Verification items for the finished model (mm, model axes). A direction names the side the tool comes from. Round coordinates to 2 decimals unless told otherwise and drop trailing zeros. Order: outer loops, then holes, each group sorted by start corner. A loop starts at its lowest first (then second) coordinate and runs counter-clockwise, first axis right, second up. Notation, with made-up numbers: (74, 39) -> (114, 39) arc R21 cw to (114, 59) -> close; hole circle Ø4 at (15, 56.5). An arc over 180 degrees is marked (long way). Return JSON: item names as keys, results as strings. Group by question number.
Item 1: Access from +Z, -Z, +X, -X, +Y, -Y to the whole of each face (thin tool, end or side, straight path). Record for faces 1 (the flat face through (28, 122, 0)), 2 (the flat face through (29, 50, -6.5)), 3 (the flat face through (70, 0, -1)).
Item 2: Sectioned sample at A-A on y = 129. Record the cut outline in (x, z), plus the area to 4 significant figures.
Item 3: Sectioned sample at B-B on x = 15. Record the cut outline in (y, z).
Item 4: Sectioned sample at C-C on x = 132. Record the cut outline in (y, z).
Item 5: Depth check by flat-ended pin: pin 1 Ø2 at (y, z) = (38, 0.5) entering from +X; pin 2 Ø3 at (x, z) = (27.5, -1) entering from -Y; pin 3 Ø13.5 at (x, y) = (15, 129) entering from -Z; pin 4 Ø6 at (y, z) = (86.5, 4) entering from +X. Enter the tip coordinate at first touch or a pass-through.
Item 6: Sectioned sample at D-D on z = 1. Record the cut outline in (x, y), plus the area to 3 significant figures.
Item 7: Draft check along X on faces 4 (the cylindrical face through (137.495, 23.758, -0.091)), 5 (the cylindrical face through (2.281, 141.594, 0.091)), 6 (the flat face through (142, 12, 0)). Enter one of: pulls with the +X half, pulls with the -X half, needs draft (parallel to the pull), parting line crosses it, or undercut.
Item 8: Scan lines: probe 1 along Y at (x, z) = (15, -0.75); probe 2 along X at (y, z) = (24, 0.75); probe 3 along Y at (x, z) = (132, 1.75). Record each from-to range of solid material in increasing order. Write a range as from..to.
```python
from build123d import *

# Parameters (mm, degrees)
SKETCH1_R           = 5.5
BOSS_EXTRUDE1_DEPTH = 6.5
SKETCH2_W           = 142
SKETCH2_H           = 7
BOSS_EXTRUDE2_DEPTH = 3
M10_TAPPED_HOLE1_D  = 8.5
FILLET1_R           = 8


with BuildPart() as part:
    # Sketch1 → Boss-Extrude1 (new, symmetric)
    with BuildSketch(Plane.XY):
        with BuildLine():
            Line((28, 144), (28, 106.83281573))
            ThreePointArc((28, 106.83281573), (46.591206617, 30.06239302), (125.561643836, 31.794678205))
            ThreePointArc((125.561643836, 31.794678205), (136.219978576, 33.209008103), (142, 24.143039825))
            Line((142, 24.143039825), (142, 0))
            Line((142, 0), (0, 0))
            Line((0, 0), (0, 144))
            Line((0, 144), (28, 144))
        make_face()
        with Locations(Location((132, 24, 0), (0, 0, 180))):
            Circle(SKETCH1_R, mode=Mode.SUBTRACT)
    extrude(amount=BOSS_EXTRUDE1_DEPTH, both=True)

    # Sketch2 → Boss-Extrude2 (add)
    with BuildSketch(Plane.XY.offset(-6.5)):
        with Locations((71, 3.5)):
            Rectangle(SKETCH2_W, SKETCH2_H)
    extrude(amount=-BOSS_EXTRUDE2_DEPTH)

    # M10 Tapped Hole1 (through all)
    with Locations(Plane.XY.offset(6.5)):
        with Locations((15, 129)):
            Hole(M10_TAPPED_HOLE1_D / 2)

    # Fillet1
    fillet1_edges = [part.edges().sort_by_distance(p)[0] for p in [
        (0, 144, 0),
        (28, 144, 0),
    ]]
    fillet(fillet1_edges, radius=FILLET1_R)


solid = part.part
```
Recorded:
{
 "1": {"face 1": "+Z, -Z, +X, +Y", "face 2": "-Z, +X, -X, +Y", "face 3": "+Z, -Z, +X, -X, -Y"},
 "2": {"outline": "(0, -6.5) -> (10.75, -6.5) -> (10.75, 6.5) -> (0, 6.5) -> close; (19.25, -6.5) -> (28, -6.5) -> (28, 6.5) -> (19.25, 6.5) -> close", "area": "253.5 mm²"},
 "3": {"outline": "(0, -9.5) -> (7, -9.5) -> (7, -6.5) -> (124.75, -6.5) -> (124.75, 6.5) -> (0, 6.5) -> close; (133.25, -6.5) -> (144, -6.5) -> (144, 6.5) -> (133.25, 6.5) -> close"},
 "4": {"outline": "(0, -9.5) -> (7, -9.5) -> (7, -6.5) -> (18.5, -6.5) -> (18.5, 6.5) -> (0, 6.5) -> close; (29.5, -6.5) -> (34.14, -6.5) -> (34.14, 6.5) -> (29.5, 6.5) -> close"},
 "5": {"pin 1": "x = 38.96", "pin 2": "y = 0", "pin 3": "z = -6.5", "pin 4": "x = 22.72"},
 "6": {"outline": "(0, 0) -> (142, 0) -> (142, 24.14) arc R10 ccw to (125.56, 31.79) arc R63 cw to (28, 106.83) -> (28, 136) arc R8 ccw to (20, 144) -> (8, 144) arc R8 ccw to (0, 136) -> close; hole circle Ø8.5 at (15, 129); hole circle Ø11 at (132, 24)", "area": "6,600 mm²"},
 "7": {"face 4": "undercut", "face 5": "pulls with the -X half", "face 6": "pulls with the +X half"},
 "8": {"probe 1": "0..124.75, 133.25..144", "probe 2": "0..56.14, 113.86..126.5, 137.5..142", "probe 3": "0..18.5, 29.5..34.14"}
}
